Input: part model. Units: mm. Frame: model coordinates. A direction names the side the tool comes from. Coordinates: 2 decimals unless noted, no trailing zeros. Loops run counter-clockwise (first coordinate to the right, second up) from the corner with the lowest first, then second, coordinate; pieces in that order, holes last.
(1) Mould query, pull axis Y, two halves, no side actions, for faces 3 (the face through (-2.38, -10.74, 6.08)), 4 (the face through (12.932, -5.362, 10.226)), 5 (the face through (-15, 0, 0)). Classes: released by +Y, released by -Y, zero draft, split by the parting line, or undercut.
(2) Section C-C, the plane z = 7.5. Return loops of the section in (x, y), then the cut area to 3 significant figures.
(3) Line query: L1, parallel to Y at x = 0, z = 1.7; L2, parallel to Y at x = 26, z = 2.05; L3, parallel to Y at x = 0, z = 3.5. Output: solid intervals per line, ascending.
(4) Contact query for flat-ended pins moving along their axis: P1, Ø4.5, axis at x = 0, y = 26, coming from the +Z side; P2, Ø1.5, axis at x = 11, z = 9.5, coming from the -Y side; P3, Ø3, axis at y = 17, z = 6.5, coming from the -X side; P4, Ø12, axis at x = -18.5, y = 14.5, coming from the +Z side. Output: stop coordinate, or through.
(5) Set-up query: faces 1 (the face through (0, -32, 1)), 2 (the face through (6, -13, 8.5)). Return all of +Z, -Z, +X, -X, +Y, -Y with unobstructed straight access to the full face (end or side cutting, diameter ignored); none if empty.
(6) Section D-D, the plane y = -7.5. Return loops of the section in (x, z).
(7) Section A-A, the plane x = 0. Return loops of the section in (y, z), then the cut area to 3 significant figures.
```python
from build123d import *

# Parameters (mm, degrees)
LUG_FLANGE_DEPTH            = 3
HUB_SKETCH_R                = 17
HUB_BOSS_DEPTH              = 5.5
SPIGOT_SKETCH_R             = 14
LOCATING_SPIGOT_DEPTH       = 3.5
BEARING_BORE_SKETCH_R       = 11
BEARING_BORE_DEPTH          = 15
LUG_HOLES_SKETCH_R          = 2.5
LUG_MOUNTING_HOLES_4X_DEPTH = 15


with BuildPart() as part:
    # Flange Profile Sketch → Lug Flange (new body)
    with BuildSketch(Plane.XY):
        with BuildLine():
            ThreePointArc((9.908335055, -20.200863755), (15.909902577, -15.909902577), (20.200863755, -9.908335055))
            ThreePointArc((20.200863755, -9.908335055), (22.672432853, -7.120669901), (26.224112426, -5.995813007))
            ThreePointArc((26.224112426, -5.995813007), (32, 0), (26.224112426, 5.995813007))
            ThreePointArc((26.224112426, 5.995813007), (22.672432853, 7.120669901), (20.200863755, 9.908335055))
            ThreePointArc((20.200863755, 9.908335055), (15.909902577, 15.909902577), (9.908335055, 20.200863755))
            ThreePointArc((9.908335055, 20.200863755), (7.120669901, 22.672432853), (5.995813007, 26.224112426))
            ThreePointArc((5.995813007, 26.224112426), (0, 32), (-5.995813007, 26.224112426))
            ThreePointArc((-5.995813007, 26.224112426), (-7.120669901, 22.672432853), (-9.908335055, 20.200863755))
            ThreePointArc((-9.908335055, 20.200863755), (-15.909902577, 15.909902577), (-20.200863755, 9.908335055))
            ThreePointArc((-20.200863755, 9.908335055), (-22.672432853, 7.120669901), (-26.224112426, 5.995813007))
            ThreePointArc((-26.224112426, 5.995813007), (-32, 0), (-26.224112426, -5.995813007))
            ThreePointArc((-26.224112426, -5.995813007), (-22.672432853, -7.120669901), (-20.200863755, -9.908335055))
            ThreePointArc((-20.200863755, -9.908335055), (-15.909902577, -15.909902577), (-9.908335055, -20.200863755))
            ThreePointArc((-9.908335055, -20.200863755), (-7.120669901, -22.672432853), (-5.995813007, -26.224112426))
            ThreePointArc((-5.995813007, -26.224112426), (0, -32), (5.995813007, -26.224112426))
            ThreePointArc((5.995813007, -26.224112426), (7.120669901, -22.672432853), (9.908335055, -20.200863755))
        make_face()
    extrude(amount=LUG_FLANGE_DEPTH)

    # Hub Sketch → Hub Boss (add)
    with BuildSketch(Plane.XY.offset(3)):
        with Locations(Location((0, 0, 0), (0, 0, 180))):
            Circle(HUB_SKETCH_R)
    extrude(amount=HUB_BOSS_DEPTH)

    # Spigot Sketch → Locating Spigot (add)
    with BuildSketch(Plane.XY.offset(8.5)):
        Circle(SPIGOT_SKETCH_R)
    extrude(amount=LOCATING_SPIGOT_DEPTH)

    # Bearing Bore Sketch → Bearing Bore (cut)
    with BuildSketch(Plane.XY.offset(12)):
        Circle(BEARING_BORE_SKETCH_R)
    extrude(amount=-BEARING_BORE_DEPTH, mode=Mode.SUBTRACT)

    # Lug Holes Sketch → Lug Mounting Holes 4x (cut)
    with BuildSketch(Plane.XY.offset(3)):
        with Locations((-26, 0)):
            Circle(LUG_HOLES_SKETCH_R)
        with Locations((0, 26)):
            Circle(LUG_HOLES_SKETCH_R)
        with Locations((26, 0)):
            Circle(LUG_HOLES_SKETCH_R)
        with Locations((0, -26)):
            Circle(LUG_HOLES_SKETCH_R)
    extrude(amount=-LUG_MOUNTING_HOLES_4X_DEPTH, mode=Mode.SUBTRACT)


solid = part.part
```
Report:
1. face 3: undercut
1. face 4: split by the parting line
1. face 5: zero draft
2. outline: circle Ø34 at (0, 0); hole circle Ø22 at (0, 0)
2. area: 528 mm2
3. L1: y = -32 to -28.5, -23.5 to -11, 11 to 23.5, 28.5 to 32
3. L2: y = -6.01 to -2.5, 2.5 to 6.01
3. L3: y = -17 to -11, 11 to 17
4. P1: passes through
4. P2: stops at y = -9.54
4. P3: stops at x = -6.98
4. P4: stops at z = 3
5. face 1: +Z, -Z, -Y
5. face 2: +Z
6. outline: (-22.14, 0) - (-8.05, 0) - (-8.05, 12) - (-11.82, 12) - (-11.82, 8.5) - (-15.26, 8.5) - (-15.26, 3) - (-22.14, 3) - close; (8.05, 0) - (22.14, 0) - (22.14, 3) - (15.26, 3) - (15.26, 8.5) - (11.82, 8.5) - (11.82, 12) - (8.05, 12) - close
7. outline: (-32, 0) - (-28.5, 0) - (-28.5, 3) - (-32, 3) - close; (-23.5, 0) - (-11, 0) - (-11, 12) - (-14, 12) - (-14, 8.5) - (-17, 8.5) - (-17, 3) - (-23.5, 3) - close; (11, 0) - (23.5, 0) - (23.5, 3) - (17, 3) - (17, 8.5) - (14, 8.5) - (14, 12) - (11, 12) - close; (28.5, 0) - (32, 0) - (32, 3) - (28.5, 3) - close
7. area: 183 mm2
